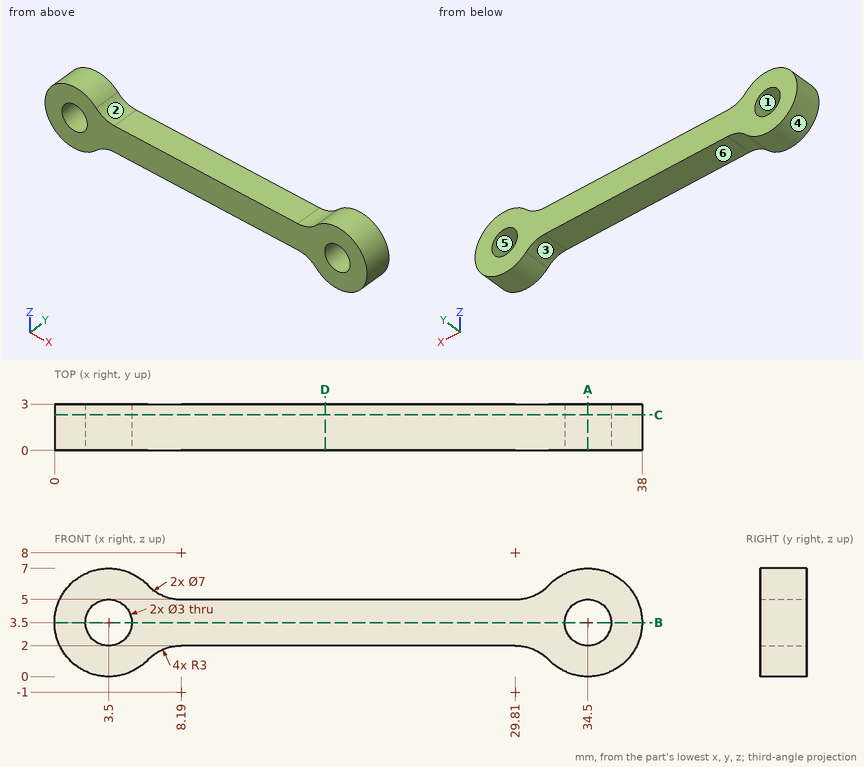
Here's the drawing with two shaded views (mm, measured from the low corner). I have some questions. A direction names the side the tool comes from. Give positions to 0.01 mm unless a question says otherwise; leave off trailing zeros. Write each loop counter-clockwise with the first axis right and the second up, starting at its lowest first coordinate (ties: lowest second). Pieces come first, ordered by that corner, then holes. Notation, with made-up numbers: (57.25, 70) -> (95.25, 70) arc R31 ccw to (95.25, 109) -> close; hole circle Ø10 at (44, -9.5). An arc over 180 degrees is marked (long way). Use one line per item in the form item = value. Start each with the question number.
1. Imagine slicing it at A-A on x = 34.5. List the corners of the cut face in (y, z) for me.
2. Imagine slicing it at C-C on y = 2.3. List the corners of the cut face in (x, z) for me (1 decimal), plus the area to 3 significant figures.
3. If I drill on L1, parallel to X at y = 2.35, z = 3.5; L2, parallel to X at y = 1.5, z = 4.75; L3, parallel to Z at x = 8, y = 2.65, over which ranges is the centre line in solid material (lowest first)?
4. Thinking about a two-plate mould opening in Z: for the marked faces 4, 5 and 6, which applies, +Z half, -Z half, draft (parallel to the pull), parting line (faces both ways), or undercut?
5. Imagine slicing it at D-D on x = 17.5. List the corners of the cut face in (y, z) for me.
6. On a 3-axis mill with a long thin cutter (end or side, diameter ignored), from which of +Z, -Z, +X, -X, +Y, -Y can I reach the whole of each face in a straight line? I mean the marked faces 1, 2 and 3. Say none if no direction works.
7. Will these pins go through, and if not, where does the flat tip stop? pin 1 Ø1 at (y, z) = (1.5, 2) entering from -X; pin 2 Ø1.5 at (y, z) = (0.5, 5) entering from +X; pin 3 Ø1.5 at (x, y) = (15.5, 1) entering from -Z; pin 4 Ø2.5 at (x, z) = (3.5, 3.5) entering from +Y.
8. Imagine slicing it at B-B on z = 3.5. List the corners of the cut face in (x, y) for me.
Entries:
q1.outline = (0, 0) -> (3, 0) -> (3, 2) -> (0, 2) -> close; (0, 5) -> (3, 5) -> (3, 7) -> (0, 7) -> close
q2.outline = (6, 1.1) arc R3 cw to (8.2, 2) -> (29.8, 2) arc R3 cw to (32, 1.1) arc R3.5 ccw (long way) to (32, 5.9) arc R3 cw to (29.8, 5) -> (8.2, 5) arc R3 cw to (6, 5.9) arc R3.5 ccw (long way) to start; hole circle Ø3 at (3.5, 3.5); hole circle Ø3 at (34.5, 3.5)
q2.area = 137 mm²
q3.L1 = 0 to 2, 5 to 33, 36 to 38
q3.L2 = 0.23 to 2.67, 4.33 to 33.67, 35.33 to 37.77
q3.L3 = 1.99 to 5.01
q4.face_4 = parting line
q4.face_5 = undercut
q4.face_6 = -Z half
q5.outline = (0, 2) -> (3, 2) -> (3, 5) -> (0, 5) -> close
q6.face_1 = +Y, -Y
q6.face_2 = +Z, +Y, -Y
q6.face_3 = -Z, +Y, -Y
q7.pin_1 = 0.15
q7.pin_2 = 37.92
q7.pin_3 = 2
q7.pin_4 = through
q8.outline = (0, 0) -> (2, 0) -> (2, 3) -> (0, 3) -> close; (5, 0) -> (33, 0) -> (33, 3) -> (5, 3) -> close; (36, 0) -> (38, 0) -> (38, 3) -> (36, 3) -> close
